```python
from build123d import *

# Parameters (mm, degrees)
SKETCH1_R           = 40
BOSS_EXTRUDE1_DEPTH = 26
SKETCH2_R           = 50
BOSS_EXTRUDE2_DEPTH = 23
SKETCH3_R           = 72.8615
BOSS_EXTRUDE3_DEPTH = 60
SKETCH4_R           = 50
BOSS_EXTRUDE4_DEPTH = 23
SKETCH6_R           = 42.5
BOSS_EXTRUDE5_DEPTH = 30
SKETCH7_R           = 40.5
BOSS_EXTRUDE6_DEPTH = 26.5
BOSS_EXTRUDE7_START = 75
SKETCH8_R           = 40
BOSS_EXTRUDE7_DEPTH = 75


with BuildPart() as part:
    # Sketch1 → Boss-Extrude1 (new body)
    with BuildSketch(Plane.XY):
        with Locations(Location((0, 0, 0), (0, 0, 180))):
            Circle(SKETCH1_R)
    extrude(amount=BOSS_EXTRUDE1_DEPTH)

    # Sketch2 → Boss-Extrude2 (add)
    with BuildSketch(Plane(origin=(0, 0, 0), x_dir=(-1, 0, 0), z_dir=(0, 0, -1))):
        Circle(SKETCH2_R)
    extrude(amount=BOSS_EXTRUDE2_DEPTH)

    # Sketch3 → Boss-Extrude3 (add)
    with BuildSketch(Plane(origin=(0, 0, -23), x_dir=(-1, 0, 0), z_dir=(0, 0, -1))):
        Circle(SKETCH3_R)
    extrude(amount=BOSS_EXTRUDE3_DEPTH)

    # Sketch4 → Boss-Extrude4 (add)
    with BuildSketch(Plane(origin=(0, 0, -83), x_dir=(-1, 0, 0), z_dir=(0, 0, -1))):
        Circle(SKETCH4_R)
    extrude(amount=BOSS_EXTRUDE4_DEPTH)

    # Sketch6 → Boss-Extrude5 (add)
    with BuildSketch(Plane(origin=(0, 0, -106), x_dir=(-1, 0, 0), z_dir=(0, 0, -1))):
        Circle(SKETCH6_R)
    extrude(amount=BOSS_EXTRUDE5_DEPTH)

    # Sketch7 → Boss-Extrude6 (add)
    with BuildSketch(Plane(origin=(0, 0, -136), x_dir=(-1, 0, 0), z_dir=(0, 0, -1))):
        Circle(SKETCH7_R)
    extrude(amount=BOSS_EXTRUDE6_DEPTH)

    # Sketch8 → Boss-Extrude7 (add)
    with BuildSketch(Plane(origin=(0, 0, -162.5), x_dir=(-1, 0, 0), z_dir=(0, 0, -1)).offset(BOSS_EXTRUDE7_START)):
        Circle(SKETCH8_R)
    extrude(amount=-BOSS_EXTRUDE7_DEPTH)


solid = part.part
```
Geometry check sheet. Reference: the model listing, model coordinates, mm. A direction names the side the tool comes from. Coordinates: 2 decimals unless noted, no trailing zeros. Loops run counter-clockwise (first coordinate to the right, second up) from the corner with the lowest first, then second, coordinate; pieces in that order, holes last.
Item 1: Access from +Z, -Z, +X, -X, +Y, -Y to the whole of each face (thin tool, end or side, straight path). Record for faces 1 (the face through (33.727, -25.861, -120.79)), 2 (the face through (39.96, -1.76, 12.82)), 3 (the face through (-67.306, -27.906, -52.58)).
Item 2: Sectioned sample at D-D, the plane z = -5.5. Record the boundary of the cut face in (x, y), then the cut area to 3 significant figures.
Item 3: Sectioned sample at C-C, the plane z = -199. Record the boundary of the cut face in (x, y).
Item 4: Go/stop test with flat-tipped pins: pin 1 Ø10 at (x, z) = (-2.5, -43) entering from +Y; pin 2 Ø6 at (y, z) = (-24.5, -167.5) entering from +X; pin 3 Ø12 at (x, z) = (-12, -70.5) entering from +Y. Record where each tip stops, or that it passes through.
Item 5: Thickness scan on line 1 (Z direction, x = -38, y = -30.5); line 2 (Z direction, x = -65, y = -24); line 3 (X direction, y = 25.5, z = -8.5). Record the ranges inside material, lowest first.
Item 6: Sectioned sample at A-A, the plane y = 0. Record the boundary of the cut face in (x, z).
Check result:
1. face 1: -Z
1. face 2: +Z
1. face 3: +Z, -Z
2. outline: circle Ø100 at (0, 0)
2. area: 7,850 mm2
3. outline: circle Ø80 at (0, 0)
4. pin 1: stops at y = 72.86
4. pin 2: stops at x = 33.73
4. pin 3: stops at y = 72.61
5. line 1: z = -106 to 0
5. line 2: z = -83 to -23
5. line 3: x = -43.01 to 43.01
6. outline: (-72.86, -83) - (-50, -83) - (-50, -106) - (-42.5, -106) - (-42.5, -136) - (-40.5, -136) - (-40.5, -162.5) - (-40, -162.5) - (-40, -237.5) - (40, -237.5) - (40, -162.5) - (40.5, -162.5) - (40.5, -136) - (42.5, -136) - (42.5, -106) - (50, -106) - (50, -83) - (72.86, -83) - (72.86, -23) - (50, -23) - (50, 0) - (40, 0) - (40, 26) - (-40, 26) - (-40, 0) - (-50, 0) - (-50, -23) - (-72.86, -23) - close
